```python
from build123d import *

# Parameters (mm, degrees)
BACK_WALL_DEPTH            = 12
BASE_PLATE_DEPTH           = 10
SQUARE_PAD_PROFILE_30X30_W = 30
SQUARE_PAD_PROFILE_30X30_H = 38
SQUARE_PAD_30X30_DEPTH     = 6
PAD_POCKET_PROFILE_W       = 16
PAD_POCKET_PROFILE_H       = 18
PAD_POCKET_DEPTH           = 10
RIB_1_DEPTH                = 20
RIB_2_DEPTH                = 20
TRIANGULAR_CUT_2_DEPTH     = 10
TRIANGULAR_CUT_1_DEPTH     = 10


with BuildPart() as part:
    # Back Wall Profile → Back Wall (new body)
    with BuildSketch(Plane.XY):
        Polygon((0, 0), (0, 48), (12, 60), (78, 60), (90, 48), (90, 0), align=None)
    extrude(amount=BACK_WALL_DEPTH)

    # Base Plate Profile → Base Plate (add)
    with BuildSketch(Plane.XZ):
        Polygon((90, 12), (0, 12), (0, 44), (6, 50), (84, 50), (90, 44), align=None)
    extrude(amount=-BASE_PLATE_DEPTH)

    # Square Pad Profile 30x30 → Square Pad 30x30 (add)
    with BuildSketch(Plane(origin=(0, 10, 0), x_dir=(1, 0, 0), z_dir=(0, 1, 0))):
        with Locations((45, -31)):
            Rectangle(SQUARE_PAD_PROFILE_30X30_W, SQUARE_PAD_PROFILE_30X30_H)
    extrude(amount=SQUARE_PAD_30X30_DEPTH)

    # Pad Pocket Profile → Pad Pocket (cut)
    with BuildSketch(Plane(origin=(0, 16, 0), x_dir=(1, 0, 0), z_dir=(0, 1, 0))):
        with Locations((45, -31)):
            Rectangle(PAD_POCKET_PROFILE_W, PAD_POCKET_PROFILE_H)
    extrude(amount=-PAD_POCKET_DEPTH, mode=Mode.SUBTRACT)

    # Rib 1 Profile → Rib 1 (add)
    with BuildSketch(Plane.ZY):
        Polygon((12, 10), (12, 42), (37, 10), align=None)
    extrude(amount=-RIB_1_DEPTH)

    # Rib 2 Profile → Rib 2 (add)
    with BuildSketch(Plane(origin=(90, 0, 0), x_dir=(0, 0, -1), z_dir=(1, 0, 0))):
        Polygon((-12, 10), (-12, 42), (-37, 10), align=None)
    extrude(amount=-RIB_2_DEPTH)

    # Triangular Cut 2 Profile → Triangular Cut 2 (cut)
    with BuildSketch(Plane(origin=(90, 0, 0), x_dir=(0, 0, -1), z_dir=(1, 0, 0))):
        Polygon((-12, 42), (-12, 10), (-37, 10), align=None)
    extrude(amount=-TRIANGULAR_CUT_2_DEPTH, mode=Mode.SUBTRACT)

    # Triangular Cut 1 Profile → Triangular Cut 1 (cut)
    with BuildSketch(Plane.ZY):
        Polygon((12, 42), (12, 10), (37, 10), align=None)
    extrude(amount=-TRIANGULAR_CUT_1_DEPTH, mode=Mode.SUBTRACT)


solid = part.part
```
The listing builds one solid part. Answer for the finished solid, in the listing's coordinates (mm). A direction names the side the tool comes from. Give positions to 0.01 mm unless a question says otherwise; leave off trailing zeros. Write each loop counter-clockwise with the first axis right and the second up, starting at its lowest first coordinate (ties: lowest second). Pieces come first, ordered by that corner, then holes. Notation, with made-up numbers: (48.5, -28.5) - (90.5, -28.5) arc R18 cw to (90.5, -20.5) - close; hole circle Ø8 at (-2, -11). An arc over 180 degrees is marked (long way). Use one line per item in the form item = value. Start each with the question number.
1) Find section A-A on z = 19.5. Determine the outline of the cut face in (x, y), plus the area to 3 significant figures.
2) The mould has two halves that part along X. Classify faces 5 (the face through (6, 54, 6)), 6 (the face through (14.93, 26.22, 24.33)), 7 (the face through (37, 11, 31)): pulls with the +X half, pulls with the -X half, needs draft (parallel to the pull), parting line crosses it, or undercut.
3) Find section D-D on z = 14. Determine the outline of the cut face in (x, y), plus the area to 3 significant figures.
4) Find section B-B on x = 16.5. Determine the outline of the cut face in (y, z), plus the area to 3 significant figures.
5) Consider line 1 along X through (y, z) = (13.5, 36.5); line 2 along Z through (x, y) = (60, 38.5); line 3 along Y through (x, z) = (86, 47). Determine where each line is inside the solid, lowest interval first. Write a range as from..to.
6) Find section C-C on y = 27. Determine the outline of the cut face in (x, z), plus the area to 3 significant figures.
7) A tool of negligible diameter and unlimited length cuts with its end or side. For faces 1 (the face through (10, 19, 19)), 2 (the face through (22, 10, 31)), 3 (the face through (80, 19, 19)), 4 (the face through (45, 11, 40)), from which of +Z, -Z, +X, -X, +Y, -Y can it reach the whole face along a straight path? Write none if from no direction.
8) Flat-ended cylindrical pins translate along their axes: pin 1 Ø1.5 at (x, y) = (57, 22.5) entering from +Z; pin 2 Ø15 at (x, z) = (15, 31) entering from +Y; pin 3 Ø24 at (x, z) = (38.5, 26) entering from +Y. Find the tip coordinate at first contact, or state that the pin passes through.
Geometry results:
q1.outline = (0, 0) - (90, 0) - (90, 10) - (80, 10) - (80, 32.4) - (70, 32.4) - (70, 10) - (60, 10) - (60, 16) - (30, 16) - (30, 10) - (20, 10) - (20, 32.4) - (10, 32.4) - (10, 10) - (0, 10) - close
q1.area = 1,530 mm2
q2.face_5 = pulls with the -X half
q2.face_6 = needs draft
q2.face_7 = undercut
q3.outline = (0, 0) - (90, 0) - (90, 10) - (80, 10) - (80, 39.44) - (70, 39.44) - (70, 10) - (60, 10) - (60, 16) - (30, 16) - (30, 10) - (20, 10) - (20, 39.44) - (10, 39.44) - (10, 10) - (0, 10) - close
q3.area = 1,670 mm2
q4.outline = (0, 0) - (60, 0) - (60, 12) - (42, 12) - (10, 37) - (10, 50) - (0, 50) - close
q4.area = 1,500 mm2
q5.line_1 = 30..37, 53..60
q5.line_2 = 0..12
q5.line_3 = 0..10
q6.outline = (0, 0) - (90, 0) - (90, 12) - (80, 12) - (80, 23.72) - (70, 23.72) - (70, 12) - (20, 12) - (20, 23.72) - (10, 23.72) - (10, 12) - (0, 12) - close
q6.area = 1,310 mm2
q7.face_1 = +Z, -X, +Y
q7.face_2 = +Z, +Y
q7.face_3 = +Z, +X, +Y
q7.face_4 = +Y
q8.pin_1 = 12
q8.pin_2 = 27.28
q8.pin_3 = 16
